```python
from build123d import *

# Parameters (mm, degrees)
EXTRUDE_1_DEPTH          = 2.5
SKETCH_4_R               = 13.05
EXTRUDE_3_DEPTH          = 12
CUT_EXTRUDE_2_REACH      = 29.921
SKETCH_5_R               = 9
SKETCH_6_R               = 14.5
SKETCH_6_R_2             = 9
EXTRUDE_4_DEPTH          = 12
HOLE_WIZARD_G3_4_1_D     = 24.5
HOLE_WIZARD_G3_4_1_DEPTH = 15
HOLE_WIZARD_G3_4_1_TIP   = 7.360542583
CHAMFER_1_SIZE           = 1


with BuildPart() as part:
    # 草图1 → 凸台-拉伸1 (new, symmetric)
    with BuildSketch(Plane.XY):
        Polygon((16.743157806, 0), (8.371578903, 14.5), (-8.371578903, 14.5), (-16.743157806, 0), (-8.371578903, -14.5), (8.371578903, -14.5), align=None)
    extrude(amount=EXTRUDE_1_DEPTH, both=True)

    # 草图4 → 凸台-拉伸3 (add)
    with BuildSketch(Plane(origin=(0, 0, -2.5), x_dir=(-1, 0, 0), z_dir=(0, 0, -1))):
        Circle(SKETCH_4_R)
    extrude(amount=EXTRUDE_3_DEPTH)

    # 草图5 → 切除-拉伸2 (cut, up to next)
    with BuildSketch(Plane(origin=(0, 0, -14.5), x_dir=(-1, 0, 0), z_dir=(0, 0, -1)), mode=Mode.PRIVATE) as cut_extrude_2_sk1:
        Circle(SKETCH_5_R)
    cut_extrude_2_tool1 = extrude(cut_extrude_2_sk1.sketch, amount=-CUT_EXTRUDE_2_REACH, mode=Mode.PRIVATE) & part.part
    add(cut_extrude_2_tool1.solids().sort_by_distance((0, 0, -14.5))[0], mode=Mode.SUBTRACT)

    # 草图6 → 凸台-拉伸4 (add)
    with BuildSketch(Plane.XY.offset(2.5)):
        with Locations(Location((0, 0, 0), (0, 0, 150))):
            Circle(SKETCH_6_R)
        with Locations(Location((0, 0, 0), (0, 0, 180))):
            Circle(SKETCH_6_R_2, mode=Mode.SUBTRACT)
    extrude(amount=EXTRUDE_4_DEPTH)

    # G3/4 螺纹孔1
    with Locations(Plane.XY.offset(14.5)):
        with Locations((0, 0)):
            Hole(HOLE_WIZARD_G3_4_1_D / 2, depth=HOLE_WIZARD_G3_4_1_DEPTH)
            with Locations((0, 0, -(HOLE_WIZARD_G3_4_1_DEPTH + HOLE_WIZARD_G3_4_1_TIP / 2))):  # 118° drill point
                Cone(0, HOLE_WIZARD_G3_4_1_D / 2, HOLE_WIZARD_G3_4_1_TIP, mode=Mode.SUBTRACT)

    # 倒角1
    chamfer_1_edges = [part.edges().sort_by_distance(p)[0] for p in [
        (13.05, 0, -14.5),
        (12.557368355, -7.25, 14.5),
    ]]
    chamfer(chamfer_1_edges, length=CHAMFER_1_SIZE)


solid = part.part
```
Geometry check sheet. Reference: the model listing, model coordinates, mm. A direction names the side the tool comes from. Give positions to 0.01 mm unless a question says otherwise; leave off trailing zeros. Write each loop counter-clockwise with the first axis right and the second up, starting at its lowest first coordinate (ties: lowest second). Pieces come first, ordered by that corner, then holes.
1) Access from +Z, -Z, +X, -X, +Y, -Y to the whole of each face (thin tool, end or side, straight path). Record for faces 1 (the flat face through (-7, 13, 2.5)), 2 (the flat face through (8, 13, 2.5)), 3 (the flat face through (15, 0, 2.5)), 4 (the cylindrical face through (9.62, 8.82, -7.92)).
2) Material ranges on L1, parallel to Y at x = 0, z = -9.5; L2, parallel to X at y = 0, z = 9, recorded low to high.
3) Release check for a two-part mould opening along Y. For faces 5 (the flat face through (-12.5, 7.35, 0.04)), 6 (the cylindrical face through (14.377, 1.888, 7.923)), 7 (the conical face through (-1.995, -8.984, -2.331)), 8 (the cylindrical face through (6.633, -6.083, -8.561)) record: pulls with the +Y half, pulls with the -Y half, needs draft (parallel to the pull), parting line crosses it, or undercut.
4) Section check B-B, the plane z = 5.75. Record the boundary of the cut face in (x, y), and give its area (3 significant figures).
5) Gauge pin test, flat ends, axial feed: pin 1 (2 mm diameter, centred on x = 4, z = -8.5, fed in from -Y); pin 2 (3.5 mm diameter, centred on x = -15.5, y = 1, fed in from +Z); pin 3 (2 mm diameter, centred on y = -6.5, z = 2, fed in from -X). Record the tip position at first contact, or that the pin passes through.
6) Section check C-C, the plane z = -10.5. Record the boundary of the cut face in (x, y).
7) Section check A-A, the plane z = -1.25. Record the boundary of the cut face in (x, y), and give its area (3 significant figures).
Computed:
1. face 1: +Z, -X, +Y
1. face 2: +Z, +X, +Y
1. face 3: +Z, +X
1. face 4: -Z
2. L1: y = -13.05 to -9, 9 to 13.05
2. L2: x = -14.5 to -12.25, 12.25 to 14.5
3. face 5: pulls with the +Y half
3. face 6: parting line crosses it
3. face 7: undercut
3. face 8: undercut
4. outline: circle Ø29 at (0, 0); hole circle Ø24.5 at (0, 0)
4. area: 189 mm2
5. pin 1: stops at y = -12.7
5. pin 2: stops at z = 14.22
5. pin 3: stops at x = -13.57
6. outline: circle Ø26.1 at (0, 0); hole circle Ø18 at (0, 0)
7. outline: (-16.74, 0) - (-8.37, -14.5) - (8.37, -14.5) - (16.74, 0) - (8.37, 14.5) - (-8.37, 14.5) - close; hole circle Ø22 at (0, 0)
7. area: 348 mm2
